from build123d import *

# Parameters (mm, degrees)
BOSS_EXTRUDE1_DEPTH = 22.5
CHAMFER1_SIZE       = 3
M4_TAPPED_HOLE1_D   = 3.3


with BuildPart() as part:
    # Sketch2 → Boss-Extrude1 (new, symmetric)
    with BuildSketch(Plane(origin=(0, 0, 0), x_dir=(0, 0, -1), z_dir=(1, 0, 0))):
        Polygon((67.5, 0), (132.5, 0), (132.5, -15), (106, -15), (106, -12), (114, -12), (114, -7), (86, -7), (86, -12), (94, -12), (94, -15), (67.5, -15), align=None)
    extrude(amount=BOSS_EXTRUDE1_DEPTH, both=True)

    # Chamfer1
    chamfer1_edges = [part.edges().sort_by_distance(p)[0] for p in [
        (0, -15, -132.5),
        (0, -15, -67.5),
    ]]
    chamfer(chamfer1_edges, length=CHAMFER1_SIZE)

    # M4 Tapped Hole1 (through all)
    with Locations(Plane(origin=(0, 0, 0), x_dir=(1, 0, 0), z_dir=(0, 1, 0))):
        with Locations((-12.5, 122.5), (12.5, 122.5), (-12.5, 77.5), (12.5, 77.5)):
            Hole(M4_TAPPED_HOLE1_D / 2)


solid = part.part
For this review, take the finished solid that the model builds, in its own axes (mm). A direction names the side the tool comes from. Round coordinates to 2 decimals unless told otherwise and drop trailing zeros. Loops run counter-clockwise (first coordinate to the right, second up) from the corner with the lowest first, then second, coordinate; pieces in that order, holes last. Notation, with made-up numbers: (20.25, 68) - (76.25, 68) arc R11 ccw to (76.25, 77) - close; hole circle Ø7 at (-19, 85.25). An arc over 180 degrees is marked (long way). Use one line per item in the form item = value.
1) Clearance check with flat-ended pins moving along their axes: P1, Ø2.5, axis at x = -7.5, y = -14, coming from the -Z side; P2, Ø0.9, axis at x = 7.5, y = -13.5, coming from the +Z side; P3, Ø2.5, axis at x = -12.5, z = -122.5, coming from the +Y side; P4, Ø2, axis at x = 5.5, z = -96.5, coming from the -Y side. State where each tip first meets the part, or that it passes through.
Solutions:
P1 = -131.75
P2 = -68.55
P3 = through
P4 = -7
2) We need section B-B on x = 12.5. Write out the cut boundary in (y, z), then the cut area to 3 significant figures.
Solutions:
outline = (-15, -129.5) - (-12, -132.5) - (0, -132.5) - (0, -124.15) - (-15, -124.15) - close; (-15, -120.85) - (0, -120.85) - (0, -79.15) - (-15, -79.15) - (-15, -94) - (-12, -94) - (-12, -86) - (-7, -86) - (-7, -114) - (-12, -114) - (-12, -106) - (-15, -106) - close; (-15, -75.85) - (0, -75.85) - (0, -67.5) - (-12, -67.5) - (-15, -70.5) - close
area = 691 mm2
3) Wall thickness on probe 1 along X at (y, z) = (-7.25, -122.5); probe 2 along Z at (x, y) = (-12.5, -4.75); probe 3 along Z at (x, y) = (-12.5, -11): over which ranges is each line inside the solid? List them lowest first.
Solutions:
probe_1 = -22.5 to -14.15, -10.85 to 10.85, 14.15 to 22.5
probe_2 = -132.5 to -124.15, -120.85 to -79.15, -75.85 to -67.5
probe_3 = -132.5 to -124.15, -120.85 to -114, -86 to -79.15, -75.85 to -67.5
4) Mouldability with a two-part tool opening along Y and no side actions: class faces 1 (the face through (0, -9, -86)), 2 (the face through (22.5, -6, -100)), 3 (the face through (-0.3, -13.5, -69)) as pulls with the +Y half, pulls with the -Y half, needs draft (parallel to the pull), parting line crosses it, or undercut.
Solutions:
face_1 = undercut
face_2 = needs draft
face_3 = pulls with the -Y half
5) We need section A-A on y = -8.5. Write out the cut boundary in (x, z), then the cut area to 3 significant figures.
Solutions:
outline = (-22.5, -132.5) - (22.5, -132.5) - (22.5, -114) - (-22.5, -114) - close; (-22.5, -86) - (22.5, -86) - (22.5, -67.5) - (-22.5, -67.5) - close; hole circle Ø3.3 at (-12.5, -122.5); hole circle Ø3.3 at (-12.5, -77.5); hole circle Ø3.3 at (12.5, -122.5); hole circle Ø3.3 at (12.5, -77.5)
area = 1,630 mm2
6) Tool access review of faces 4 (the face through (0, -13, -94)), 5 (the face through (0, -10, -114)), 6 (the face through (-22.5, -6, -100)): name each direction out of +Z, -Z, +X, -X, +Y, -Y from which nothing blocks a thin tool from reaching the whole face with its end or side.
Solutions:
face_4 = +X, -X, -Y
face_5 = +X, -X
face_6 = +Z, -Z, -X, +Y, -Y
7) We need section C-C on z = -122.5. Write out the cut boundary in (x, y).
Solutions:
outline = (-22.5, -15) - (-14.15, -15) - (-14.15, 0) - (-22.5, 0) - close; (-10.85, -15) - (10.85, -15) - (10.85, 0) - (-10.85, 0) - close; (14.15, -15) - (22.5, -15) - (22.5, 0) - (14.15, 0) - close
8) We need section D-D on y = -13.5. Write out the cut boundary in (x, z).
Solutions:
outline = (-22.5, -131) - (22.5, -131) - (22.5, -106) - (-22.5, -106) - close; (-22.5, -94) - (22.5, -94) - (22.5, -69) - (-22.5, -69) - close; hole circle Ø3.3 at (-12.5, -122.5); hole circle Ø3.3 at (-12.5, -77.5); hole circle Ø3.3 at (12.5, -122.5); hole circle Ø3.3 at (12.5, -77.5)
